Geometry: final body of the model. Coordinates: model frame, mm. A direction names the side the tool comes from. Give positions to 0.01 mm unless a question says otherwise; leave off trailing zeros. Write each loop counter-clockwise with the first axis right and the second up, starting at its lowest first coordinate (ties: lowest second). Pieces come first, ordered by that corner, then holes. Notation, with made-up numbers: (76, 63) -> (130, 63) arc R17 cw to (130, 77) -> close; hole circle Ø6 at (86, -13.75). An arc over 180 degrees is marked (long way). Answer as a JSON object with one key per item and string values.
from build123d import *

# Parameters (mm, degrees)
BOSS_EXTRUDE1_DEPTH = 210


with BuildPart() as part:
    # Sketch1 → Boss-Extrude1 (new body)
    with BuildSketch(Plane.XY):
        with BuildLine():
            Line((0, 0), (30, 0))
            Line((30, 0), (30, 1))
            ThreePointArc((30, 1), (29.414213562, 2.414213562), (28, 3))
            Line((28, 3), (5, 3))
            ThreePointArc((5, 3), (3.585786438, 3.585786438), (3, 5))
            Line((3, 5), (3, 28))
            ThreePointArc((3, 28), (2.414213562, 29.414213562), (1, 30))
            Line((1, 30), (0, 30))
            Line((0, 30), (0, 0))
        make_face()
    extrude(amount=BOSS_EXTRUDE1_DEPTH)


solid = part.part
Q1. Cut plane A-A (z = 113.5). Return the cut outline in (x, y), and give its area (3 significant figures).
Values:
{"outline": "(0, 0) -> (30, 0) -> (30, 1) arc R2 ccw to (28, 3) -> (5, 3) arc R2 cw to (3, 5) -> (3, 28) arc R2 ccw to (1, 30) -> (0, 30) -> close", "area": "170 mm²"}
Q2. First-contact query: P1, Ø1.5, axis at x = 18.5, z = 112, coming from the +Y side. Flat tip, straight axial feed; report the tip coordinate or a pass-through.
Values:
{"P1": "y = 3"}
Q3. Cut plane B-B (y = 13.5). Return the cut outline in (x, z), and give its area (3 significant figures).
Values:
{"outline": "(0, 0) -> (3, 0) -> (3, 210) -> (0, 210) -> close", "area": "630 mm²"}
Q4. Set-up query: faces 1 (the flat face through (17, 3, 104)), 2 (the flat face through (2.7, 9.5, 210)). Return all of +Z, -Z, +X, -X, +Y, -Y with unobstructed straight access to the full face (end or side cutting, diameter ignored); none if empty.
Values:
{"face 1": "+Z, -Z, +X, +Y", "face 2": "+Z, +X, -X, +Y, -Y"}
Q5. Material intervals for L1, parallel to X at y = 18.5, z = 48.5; L2, parallel to Y at x = 2, z = 45, sorted ascending. Write a range as from..to.
Values:
{"L1": "0..3", "L2": "0..29.73"}
